from build123d import *

# Parameters (mm, degrees)
SKETCH1_W               = 30
SKETCH1_H               = 30
BOSS_EXTRUDE1_DEPTH     = 400
SKETCH2_W               = 24
SKETCH2_H               = 24
CUT_EXTRUDE1_DEPTH      = 492
CUT_EXTRUDE3_DEPTH      = 402.958781438
CUT_EXTRUDE6_DEPTH      = 402.958781438
CUT_EXTRUDE7_DEPTH      = 402.958781438
CUT_EXTRUDE7_DEPTH_BACK = 402.958781438
SKETCH11_R              = 3


with BuildPart() as part:
    # Sketch1 → Boss-Extrude1 (new body)
    with BuildSketch(Plane.XY):
        with Locations((-30.141748722, 10.901003365)):
            Rectangle(SKETCH1_W, SKETCH1_H)
    extrude(amount=BOSS_EXTRUDE1_DEPTH)

    # Sketch2 → Cut-Extrude1 (cut)
    with BuildSketch(Plane.XY.offset(400)):
        with Locations((-30.141748722, 10.901003365)):
            Rectangle(SKETCH2_W, SKETCH2_H)
    extrude(amount=-CUT_EXTRUDE1_DEPTH, mode=Mode.SUBTRACT)

    # Sketch4 → Cut-Extrude3 (cut, through all)
    with BuildSketch(Plane(origin=(-15.141748722, 0, 0), x_dir=(0, 0, -1), z_dir=(1, 0, 0))):
        Polygon((0, 25.901003365), (-30, -4.098996635), (0, -4.098996635), align=None)
    extrude(amount=-CUT_EXTRUDE3_DEPTH, mode=Mode.SUBTRACT)

    # Sketch8 → Cut-Extrude6 (cut, through all)
    with BuildSketch(Plane(origin=(-15.141748722, 0, 0), x_dir=(0, 0, -1), z_dir=(1, 0, 0))):
        Polygon((-400, 25.901003365), (-370, -4.098996635), (-400, -4.098996635), align=None)
    extrude(amount=-CUT_EXTRUDE6_DEPTH, mode=Mode.SUBTRACT)

    # Sketch11 → Cut-Extrude7 (cut, two sides: drawn at the far end of the back side and taken through both)
    with BuildSketch(Plane(origin=(-15.141748722, 0, 0), x_dir=(0, 0, -1), z_dir=(1, 0, 0)).offset(-CUT_EXTRUDE7_DEPTH_BACK)):
        with Locations((-330, 8.401003365)):
            Circle(SKETCH11_R)
        with Locations((-66, 8.401003365)):
            Circle(SKETCH11_R)
    extrude(amount=CUT_EXTRUDE7_DEPTH + CUT_EXTRUDE7_DEPTH_BACK, mode=Mode.SUBTRACT)


solid = part.part
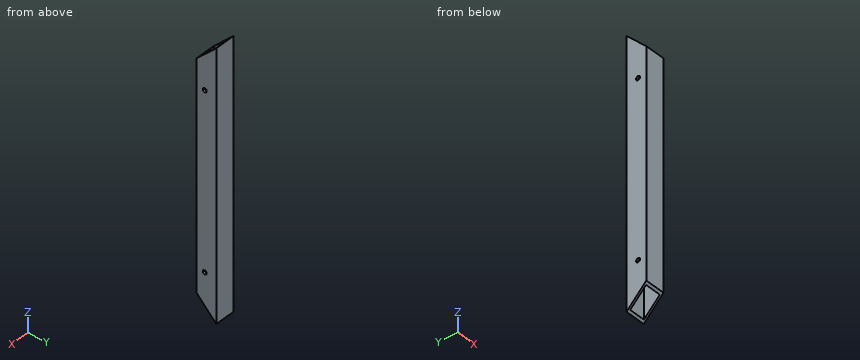
The listing builds one solid part. Answer for the finished solid, in the listing's coordinates (mm). Give positions to 0.01 mm unless a question says otherwise; leave off trailing zeros. Loops run counter-clockwise (first coordinate to the right, second up) from the corner with the lowest first, then second, coordinate; pieces in that order, holes last. Notation, with made-up numbers: M 25,0 L 40,0 A19 cw 40,25 Z; hole C 64,51.5 d5. An arc over 180 degrees is marked long. Answer as CSV lines item,"result".
Item 1: The part is cut by section C-C (y = 15.5). Give the vertices of the cut face in (x, z), and give its area (3 significant figures).
Values follow:
outline,"M -45.14,10.4 L -42.14,10.4 L -42.14,389.6 L -45.14,389.6 Z; M -18.14,10.4 L -15.14,10.4 L -15.14,389.6 L -18.14,389.6 Z"
area,"2,280 mm^2"
Item 2: The part is cut by section A-A (x = -29.5). Give the vertices of the cut face in (y, z).
Values follow:
outline,"M -4.1,30 L -1.1,27 L -1.1,373 L -4.1,370 Z; M 22.9,3 L 25.9,0 L 25.9,400 L 22.9,397 Z"
Item 3: The part is cut by section B-B (z = 50). Give the vertices of the cut face in (x, y), and give its area (3 significant figures).
Values follow:
outline,"M -45.14,-4.1 L -15.14,-4.1 L -15.14,25.9 L -45.14,25.9 Z; hole M -42.14,-1.1 L -18.14,-1.1 L -18.14,22.9 L -42.14,22.9 Z"
area,"324 mm^2"
Item 4: Given pin 1 Ø5 at (y, z) = (8.4, 66) entering from -X, flat-ended and moving along its own axis, determine where the tip first touches the part or whether it passes through.
Values follow:
pin 1,"passes through"
Item 5: Straight lines are drawn through the part: line 1 along X through (y, z) = (6, 332); line 2 along Y through (x, z) = (-16.8, 330); line 3 along Y through (x, z) = (-35.5, 261). For each, find the intervals that lie inside material, in ascending order. Write a range as [from, to].
Values follow:
line 1,"x = [-45.14, -42.14], [-18.14, -15.14]"
line 2,"y = [-4.1, 5.4], [11.4, 25.9]"
line 3,"y = [-4.1, -1.1], [22.9, 25.9]"
